```python
from build123d import *


with BuildPart() as part:
    # 草图1 → 旋转1 (revolve)
    with BuildSketch(Plane.XY, mode=Mode.PRIVATE) as revolve_1_sk:
        Polygon((0, 0), (-6, 0), (-6, 3), (-2.5, 3), (-2.5, 6.5), (-6, 6.5), (-6, 15), (0, 15), (0, 12.5), (-3.5, 12.5), (-3.5, 10.5), (0, 10.5), align=None)
    revolve(revolve_1_sk.sketch.rotate(Axis((34, 0, 0), (0, 1, 0)), 270), axis=Axis((34, 0, 0), (0, 1, 0)))


solid = part.part
```
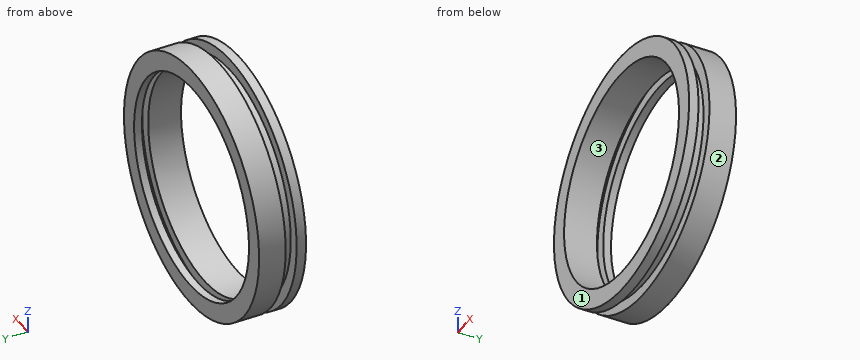
Can you work these out from the model? Positions are in its coordinate system, mm. Face numbers are marked on the shaded views. Round coordinates to 2 decimals unless told otherwise and drop trailing zeros. Loops run counter-clockwise (first coordinate to the right, second up) from the corner with the lowest first, then second, coordinate; pieces in that order, holes last. Notation, with made-up numbers: M -16.75,-15 L -1.75,-15 A30 cw -1.75,9 Z; hole C 76.5,31 d8. An arc over 180 degrees is marked long. Answer as a JSON object with one key per item and string values. Group by question number.
Q1. We'd pull the mould along X, two halves only. Please class the marked faces 1, 2 and 3: +X half, -X half, draft (parallel to the pull), parting line (faces both ways), or undercut.
Q2. Imagine slicing it at D-D, the plane y = 5.5. Please give me the cut outline in (x, z), then the cut area to 3 significant figures.
Q3. Will these pins go through, and if not, where does the flat tip stop? pin 1 (6 mm diameter, centred on x = 23.5, y = 10, fed in from -Z); pin 2 (6 mm diameter, centred on x = 22, y = 11.5, fed in from -Z); pin 3 (2 mm diameter, centred on x = 17, y = 12.5, fed in from -Z); pin 4 (22.5 mm diameter, centred on x = 50, z = -13, fed in from -Y).
Q4. Imagine slicing it at C-C, the plane y = 13.5. Please give me the cut outline in (x, z), then the cut area to 3 significant figures.
Q5. Please list where these lines run through material, in increasing order: L1, parallel to Y at x = 10.5, z = 29; L2, parallel to X at y = 14.25, z = 0; L3, parallel to X at y = 4, z = 1.
Q6. Imagine slicing it at A-A, the plane x = 34. Please give me the cut outline in (y, z), then the cut area to 4 significant figures.
Q7. Imagine slicing it at B-B, the plane z = 0. Please give me the cut outline in (x, y).
Findings:
{
 "1": {"face 1": "draft", "face 2": "parting line", "face 3": "undercut"},
 "2": {"outline": "C 34,0 d73; hole C 34,0 d68", "area": "554 mm2"},
 "3": {"pin 1": "stops at z = -39.29", "pin 2": "stops at z = -38.97", "pin 3": "stops at z = -36.66", "pin 4": "passes through"},
 "4": {"outline": "C 34,0 d80; hole C 34,0 d68", "area": "1,390 mm2"},
 "5": {"L1": "y = 0 to 3, 6.5 to 10.5, 12.5 to 15", "L2": "x = -6 to 0, 68 to 74", "L3": "x = -2.49 to 0.01, 67.99 to 70.49"},
 "6": {"outline": "M 0,-40 L 3,-40 L 3,-36.5 L 6.5,-36.5 L 6.5,-40 L 15,-40 L 15,-34 L 12.5,-34 L 12.5,-37.5 L 10.5,-37.5 L 10.5,-34 L 0,-34 Z; M 0,34 L 10.5,34 L 10.5,37.5 L 12.5,37.5 L 12.5,34 L 15,34 L 15,40 L 6.5,40 L 6.5,36.5 L 3,36.5 L 3,40 L 0,40 Z", "area": "141.5 mm2"},
 "7": {"outline": "M -6,0 L 0,0 L 0,10.5 L -3.5,10.5 L -3.5,12.5 L 0,12.5 L 0,15 L -6,15 L -6,6.5 L -2.5,6.5 L -2.5,3 L -6,3 Z; M 68,0 L 74,0 L 74,3 L 70.5,3 L 70.5,6.5 L 74,6.5 L 74,15 L 68,15 L 68,12.5 L 71.5,12.5 L 71.5,10.5 L 68,10.5 Z"}
}
